```python
from build123d import *

# Parameters (mm, degrees)
BOSS_EXTRUDE2_DEPTH = 110
SHELL2_T            = -3


with BuildPart() as part:
    # Sketch1 → Boss-Extrude2 (new body)
    with BuildSketch(Plane.XY):
        with BuildLine():
            Line((-199.186622288, 18.019142639), (-249.430635602, -537.386600152))
            ThreePointArc((-249.430635602, -537.386600152), (-217.511368505, -639.673327373), (-122.613399848, -689.430635602))
            Line((-122.613399848, -689.430635602), (735.059712531, -767.018848969))
            Line((735.059712531, -767.018848969), (759.356160444, -498.441842272))
            ThreePointArc((759.356160444, -498.441842272), (745.466568798, -405.15643604), (690.371143367, -328.608530331))
            Line((690.371143367, -328.608530331), (130.201605211, 151.814169301))
            ThreePointArc((130.201605211, 151.814169301), (-75.266263592, 185.297030642), (-199.186622288, 18.019142639))
        make_face()
    extrude(amount=BOSS_EXTRUDE2_DEPTH)

    # Shell2
    shell2_openings = [part.faces().sort_by_distance(p)[0] for p in [
        (206.21225605, -348.127169203, 0),
    ]]
    offset(amount=SHELL2_T, openings=shell2_openings, kind=Kind.INTERSECTION)


solid = part.part
```
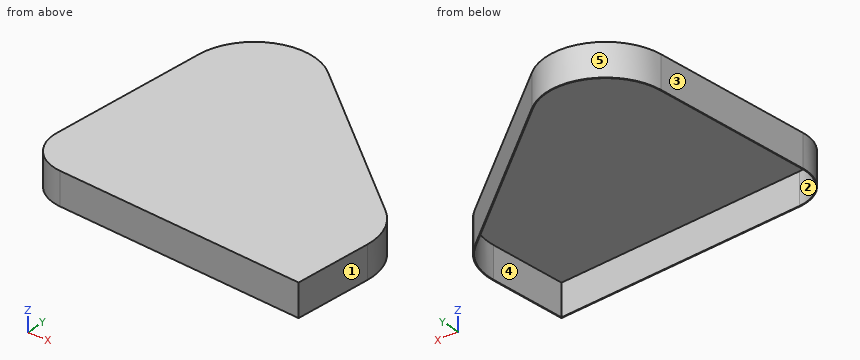
Check sheet for the modelled part. Datum: model origin and axes. Units: mm. Face numbers are marked on the shaded views. A direction names the side the tool comes from. Round coordinates to 2 decimals unless told otherwise and drop trailing zeros. Order: outer loops, then holes, each group sorted by start corner. A loop starts at its lowest first (then second) coordinate and runs counter-clockwise, first axis right, second up.
1) Section check C-C (y = -175). Record the boundary of the cut face in (x, z).
2) Section check B-B (x = 297). Record the boundary of the cut face in (y, z), and give its area (3 significant figures).
3) Tool access check on the marked faces 4 and 5. Record the directions out of +Z, -Z, +X, -X, +Y, -Y that give a thin tool (end or side, any length) a straight path to the whole face; none if there is none.
4) Section check A-A (z = 54.5). Record the boundary of the cut face in (x, y), and give its area (3 significant figures).
5) Go/stop test with flat-tipped pins: pin 1 Ø10 at (x, z) = (112, 46.5) entering from +Y; pin 2 Ø1.5 at (x, y) = (398, -105.5) entering from -Z; pin 3 Ø3 at (x, z) = (342, 71.5) entering from +Y. Record where each tip stops, or that it passes through.
6) Mould release check, pull along X, two halves, no side actions. Record for the marked faces 1, 2 and 3: +X half, -X half, draft (parallel to the pull), parting line (faces both ways), or undercut.
7) Scan lines: line 1 (Z direction, x = 263, y = -470); line 2 (Y direction, x = 22, z = 79); line 3 (Y direction, x = 408.5, z = 71). Record each from-to range of solid material in increasing order.
Result:
1. outline: (-216.65, 0) - (-213.64, 0) - (-213.64, 107) - (506.66, 107) - (506.66, 0) - (511.26, 0) - (511.26, 110) - (-216.65, 110) - close
2. outline: (-727.39, 0) - (-724.38, 0) - (-724.38, 107) - (4.81, 107) - (4.81, 0) - (8.76, 0) - (8.76, 110) - (-727.39, 110) - close
2. area: 2,950 mm2
3. face 4: -Z
3. face 5: +Z, -Z, +Y
4. outline: (-249.43, -537.39) arc R140 ccw to (-122.61, -689.43) - (735.06, -767.02) - (759.36, -498.44) arc R200 ccw to (690.37, -328.61) - (130.2, 151.81) arc R200 ccw to (-199.19, 18.02) - close; hole (-246.44, -537.66) arc R137 ccw to (-122.34, -686.44) - (732.34, -763.76) - (756.37, -498.17) arc R197 ccw to (688.42, -330.89) - (128.25, 149.54) arc R197 ccw to (-196.2, 17.75) - close
4. area: 9,790 mm2
5. pin 1: stops at y = 168.97
5. pin 2: stops at z = 107
5. pin 3: stops at y = -28.55
6. face 1: +X half
6. face 2: undercut
6. face 3: -X half
7. line 1: z = 107 to 110
7. line 2: y = -702.51 to -699.5, 195.77 to 198.79
7. line 3: y = -737.48 to -734.46, -90.82 to -86.87
